The model under review builds one solid part; all positions refer to its coordinate system, in mm. Give positions to 0.01 mm unless a question says otherwise; leave off trailing zeros. Loops run counter-clockwise (first coordinate to the right, second up) from the corner with the lowest first, then second, coordinate; pieces in that order, holes last. Notation, with made-up numbers: M 44,-14 L 95,-14 A23 ccw 95,25 Z; hole C 86.25,22 d8. An arc over 180 degrees is marked long. Return JSON: item names as keys, results as strings.
```python
from build123d import *

# Parameters (mm, degrees)
EXTRUDE_1_DEPTH = 8
CHAMFER_1_SIZE  = 15


with BuildPart() as part:
    # 草图1 → 凸台-拉伸1 (new body)
    with BuildSketch(Plane.XY):
        Polygon((0, 0), (100, 0), (100, 15), (15, 110), (0, 110), align=None)
    extrude(amount=EXTRUDE_1_DEPTH)

    # 倒角1
    chamfer_1_edges = [part.edges().sort_by_distance(p)[0] for p in [
        (0, 0, 4),
    ]]
    chamfer(chamfer_1_edges, length=CHAMFER_1_SIZE)


solid = part.part
```
1) Consider section A-A on z = 4.75. Write out the cut boundary in (x, y).
From the geometry:
{"outline": "M 0,15 L 15,0 L 100,0 L 100,15 L 15,110 L 0,110 Z"}
2) Consider section B-B on y = 89. Write out the cut boundary in (x, z), then the cut area to 3 significant figures.
From the geometry:
{"outline": "M 0,0 L 33.79,0 L 33.79,8 L 0,8 Z", "area": "270 mm²"}
3) Wall thickness on L1, parallel to X at y = 100.5, z = 0.75; L2, parallel to Y at x = 82, z = 1.5; L3, parallel to X at y = 32.5, z = 1.75: over which ranges is each line inside the solid? List them lowest first. Write a range as from..to.
From the geometry:
{"L1": "0..23.5", "L2": "0..35.12", "L3": "0..84.34"}
4) The part is to be moulded in two halves that separate along Y. For faces 1 (the face through (58.09, 61.84, 3.94)), 2 (the face through (57, 0, 4)), 3 (the face through (38, 44, 8)), say which applies: released by +Y, released by -Y, zero draft, split by the parting line, or undercut.
From the geometry:
{"face 1": "released by +Y", "face 2": "released by -Y", "face 3": "zero draft"}
5) Consider section C-C on x = 64. Write out the cut boundary in (y, z).
From the geometry:
{"outline": "M 0,0 L 55.24,0 L 55.24,8 L 0,8 Z"}
